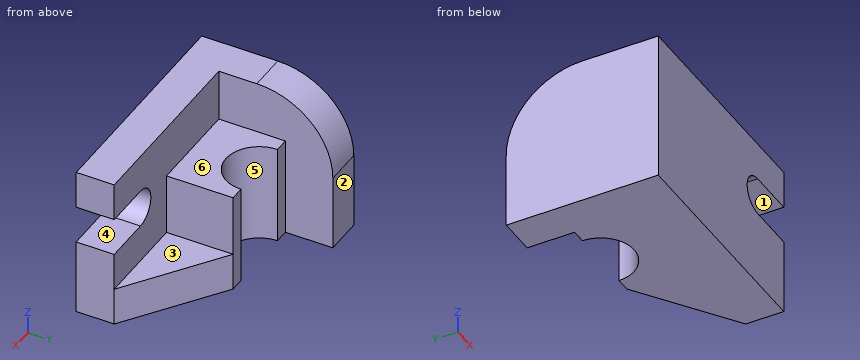
```python
from build123d import *

# Parameters (mm, degrees)
BASE_PLATE_SKETCH_W         = 96
BASE_PLATE_SKETCH_H         = 64
BASE_PLATE_96X64X16_DEPTH   = 16
U_SLOT_DEPTH                = 16
UPRIGHT_R32_DEPTH           = 16
CRADLE_BLOCK_SKETCH_W       = 40
CRADLE_BLOCK_SKETCH_H       = 42
CRADLE_BLOCK_40X22X28_DEPTH = 28
CRADLE_BORE_SKETCH_R        = 14
CRADLE_BORE_28_DEPTH        = 123.784363825
GUSSET_RIB_DEPTH            = 16


with BuildPart() as part:
    # Base Plate Sketch → Base Plate 96x64x16 (new body)
    with BuildSketch(Plane(origin=(0, 0, 0), x_dir=(1, 0, 0), z_dir=(0, 1, 0))):
        with Locations((48, 32)):
            Rectangle(BASE_PLATE_SKETCH_W, BASE_PLATE_SKETCH_H)
    extrude(amount=BASE_PLATE_96X64X16_DEPTH)

    # U-Slot Sketch → U-Slot (cut)
    with BuildSketch(Plane(origin=(0, 16, 0), x_dir=(1, 0, 0), z_dir=(0, 1, 0))):
        with BuildLine():
            Line((96, 16), (76, 16))
            ThreePointArc((76, 16), (68, 24), (76, 32))
            Line((76, 32), (96, 32))
            ThreePointArc((96, 32), (104, 24), (96, 16))
        make_face()
    extrude(amount=-U_SLOT_DEPTH, mode=Mode.SUBTRACT)

    # Upright Sketch → Upright R32 (add)
    with BuildSketch(Plane.ZY):
        with BuildLine():
            Line((-64, 0), (0, 0))
            Line((0, 0), (0, 32))
            ThreePointArc((0, 32), (-9.372583002, 54.627416998), (-32, 64))
            Line((-32, 64), (-64, 64))
            Line((-64, 64), (-64, 0))
        make_face()
    extrude(amount=-UPRIGHT_R32_DEPTH)

    # Cradle Block Sketch → Cradle Block 40x22x28 (add)
    with BuildSketch(Plane(origin=(0, 16, 0), x_dir=(1, 0, 0), z_dir=(0, 1, 0))):
        with Locations((36, 43)):
            Rectangle(CRADLE_BLOCK_SKETCH_W, CRADLE_BLOCK_SKETCH_H)
    extrude(amount=CRADLE_BLOCK_40X22X28_DEPTH)

    # Cradle Bore Sketch → Cradle Bore Ø28 (cut, through all)
    with BuildSketch(Plane.XY.offset(-22)):
        with Locations((36, 44)):
            Circle(CRADLE_BORE_SKETCH_R)
    extrude(amount=-CRADLE_BORE_28_DEPTH, mode=Mode.SUBTRACT)

    # Gusset Rib Sketch → Gusset Rib (add)
    with BuildSketch(Plane(origin=(0, 0, -64), x_dir=(-1, 0, 0), z_dir=(0, 0, -1))):
        Polygon((-56, 44), (-56, 16), (-96, 16), align=None)
    extrude(amount=-GUSSET_RIB_DEPTH)


solid = part.part
```
Could you check a few things on this model? Use its own coordinates, in mm. Face numbers are marked on the shaded views. A direction names the side the tool comes from. Round coordinates to 2 decimals unless told otherwise and drop trailing zeros. Loops run counter-clockwise (first coordinate to the right, second up) from the corner with the lowest first, then second, coordinate; pieces in that order, holes last. Notation, with made-up numbers: (-6, -17.75) - (31, -17.75) arc R14 cw to (31, 6.25) - close; hole circle Ø7 at (68.5, 21.5). An arc over 180 degrees is marked (long way). Answer as CSV lines item,"result".
1. I want a section at D-D on z = -52.5. List the corners of the cut face in (x, y) for me.
Filled in:
outline,"(0, 0) - (96, 0) - (96, 16) - (56, 44) - (50, 44) arc R14 cw to (22, 44) - (16, 44) - (16, 64) - (0, 64) - close"
2. For pin 1 Ø6 at (x, z) = (73, -21) entering from +Y; pin 2 Ø2 at (x, y) = (13, 40.5) entering from +Z; pin 3 Ø4 at (x, z) = (26.5, -16.5) entering from +Y; pin 4 Ø6.5 at (x, z) = (52.5, -53) entering from +Y, each with a flat end and sliding along its axis, tell me the tip position at first contact or that it passes through.
Filled in:
pin 1,"passes through"
pin 2,"stops at z = -0.89"
pin 3,"stops at y = 16"
pin 4,"stops at y = 44"
3. Please list where these lines run through material, in increasing order: line 1 along Y through (x, z) = (55, -42); line 2 along X through (y, z) = (23, -30.5); line 3 along Z through (x, y) = (64.5, 24). Write a range as [from, to].
Filled in:
line 1,"y = [0, 44]"
line 2,"x = [0, 56]"
line 3,"z = [-64, -48]"
4. On a 3-axis mill with a long thin cutter (end or side, diameter ignored), from which of +Z, -Z, +X, -X, +Y, -Y can I reach the whole of each face in a straight line? I mean the marked faces 1, 2 and 3. Say none if no direction works.
Filled in:
face 1,"+X, +Y, -Y"
face 2,"+Z, -Z, +X, -X, +Y"
face 3,"+Z, +X, +Y"
5. I want a section at A-A on x = 90.5. List the corners of the cut face in (y, z) for me, then the cut area to 3 significant figures.
Filled in:
outline,"(0, -64) - (19.85, -64) - (19.85, -48) - (16, -48) - (16, -32) - (0, -32) - close; (0, -16) - (16, -16) - (16, 0) - (0, 0) - close"
area,"830 mm^2"
6. I want a section at C-C on y = 7. List the corners of the cut face in (x, z) for me, then the cut area to 3 significant figures.
Filled in:
outline,"(0, -64) - (96, -64) - (96, -32) - (76, -32) arc R8 cw to (76, -16) - (96, -16) - (96, 0) - (0, 0) - close"
area,"5,720 mm^2"
7. We'd pull the mould along Z, two halves only. Please class the marked faces 4, 5 and 6: +Z half, -Z half, draft (parallel to the pull), parting line (faces both ways), or undercut.
Filled in:
face 4,"undercut"
face 5,"draft"
face 6,"+Z half"
8. I want a section at B-B on y = 38.5. List the corners of the cut face in (x, z) for me.
Filled in:
outline,"(0, -64) - (23.13, -64) - (23.13, -22) - (16, -22) - (16, -0.67) - (0, -0.67) - close; (48.87, -64) - (63.86, -64) - (63.86, -48) - (56, -48) - (56, -22) - (48.87, -22) - close"
